Verification items for the finished model (mm, model axes). Face numbers are marked on the shaded views. A direction names the side the tool comes from. Give positions to 0.01 mm unless a question says otherwise; leave off trailing zeros. Write each loop counter-clockwise with the first axis right and the second up, starting at its lowest first coordinate (ties: lowest second). Pieces come first, ordered by that corner, then holes. Notation, with made-up numbers: (86.5, 28.5) -> (112.5, 28.5) arc R16 ccw to (112.5, 36.5) -> close; hole circle Ø11 at (42, 70). An arc over 180 degrees is marked (long way). Use one line per item in the form item = value. Start each with the question number.
(1) Depth check by flat-ended pin: pin 1 Ø5 at (x, z) = (-81.5, -1) entering from +Y; pin 2 Ø5 at (x, z) = (-165, 0) entering from -Y; pin 3 Ø4 at (y, z) = (6.5, -2) entering from +X; pin 4 Ø8 at (x, y) = (38.5, 14.5) entering from +Z. Enter the tip coordinate at first touch or a pass-through.
(2) Scan lines: L1, parallel to Z at x = -165, y = 1.9; L2, parallel to Z at x = -152, y = 7.75; L3, parallel to Y at x = -102, z = -3. Record each from-to range of solid material in increasing order.
(3) Section check C-C, the plane y = 12.25. Record the cut outline in (x, z), plus the area to 3 significant figures.
(4) Section check A-A, the plane z = 0. Record the cut outline in (x, y), plus the area to 3 significant figures.
(5) Section check B-B, the plane x = 64. Record the cut outline in (y, z).
(6) Set-up check for the marked faces 1 and 2: record each of +Z, -Z, +X, -X, +Y, -Y from which the full face is reachable in a straight line by a thin tool's end or side.
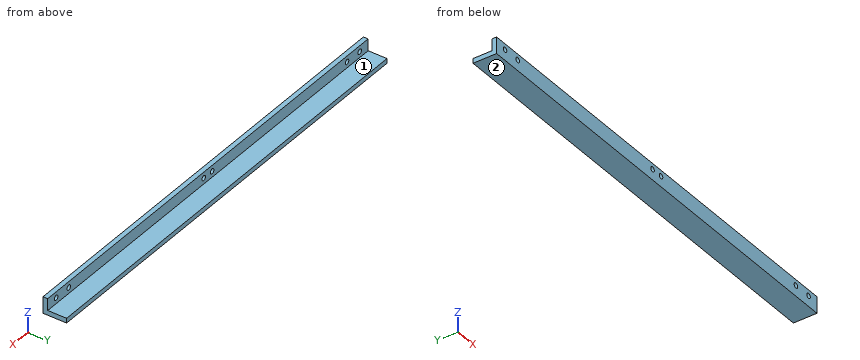
from build123d import *

# Parameters (mm, degrees)
SKETCH1_W           = 380
SKETCH1_H           = 10
SKETCH1_R           = 2.1
BOSS_EXTRUDE1_DEPTH = 4
SKETCH2_W           = 380
SKETCH2_H           = 20
BOSS_EXTRUDE2_DEPTH = 4


with BuildPart() as part:
    # Sketch1 → Boss-Extrude1 (new body)
    with BuildSketch(Plane(origin=(0, 0, 0), x_dir=(1, 0, 0), z_dir=(0, 1, 0))):
        Rectangle(SKETCH1_W, SKETCH1_H)
        with Locations(Location((-180, 0, 0), (0, 0, 270))):
            Circle(SKETCH1_R, mode=Mode.SUBTRACT)
        with Locations(Location((-165, 0, 0), (0, 0, 270))):
            Circle(SKETCH1_R, mode=Mode.SUBTRACT)
        with Locations(Location((165, 0, 0), (0, 0, 90))):
            Circle(SKETCH1_R, mode=Mode.SUBTRACT)
        with Locations(Location((180, 0, 0), (0, 0, 90))):
            Circle(SKETCH1_R, mode=Mode.SUBTRACT)
        with Locations(Location((5, 0, 0), (0, 0, 270))):
            Circle(SKETCH1_R, mode=Mode.SUBTRACT)
        with Locations(Location((-5, 0, 0), (0, 0, 270))):
            Circle(SKETCH1_R, mode=Mode.SUBTRACT)
    extrude(amount=BOSS_EXTRUDE1_DEPTH)

    # Sketch2 → Boss-Extrude2 (add)
    with BuildSketch(Plane(origin=(0, 0, -5), x_dir=(-1, 0, 0), z_dir=(0, 0, -1))):
        with Locations((0, 10)):
            Rectangle(SKETCH2_W, SKETCH2_H)
    extrude(amount=BOSS_EXTRUDE2_DEPTH)


solid = part.part
Completed:
q1.pin_1 = 4
q1.pin_2 = 0
q1.pin_3 = through
q1.pin_4 = -5
q2.L1 = -9 to -2.1, 2.1 to 5
q2.L2 = -9 to -5
q2.L3 = 0 to 4
q3.outline = (-190, -9) -> (190, -9) -> (190, -5) -> (-190, -5) -> close
q3.area = 1,520 mm²
q4.outline = (-190, 0) -> (-182.1, 0) -> (-182.1, 4) -> (-190, 4) -> close; (-177.9, 0) -> (-167.1, 0) -> (-167.1, 4) -> (-177.9, 4) -> close; (-162.9, 0) -> (-7.1, 0) -> (-7.1, 4) -> (-162.9, 4) -> close; (-2.9, 0) -> (2.9, 0) -> (2.9, 4) -> (-2.9, 4) -> close; (7.1, 0) -> (162.9, 0) -> (162.9, 4) -> (7.1, 4) -> close; (167.1, 0) -> (177.9, 0) -> (177.9, 4) -> (167.1, 4) -> close; (182.1, 0) -> (190, 0) -> (190, 4) -> (182.1, 4) -> close
q4.area = 1,420 mm²
q5.outline = (0, -9) -> (20, -9) -> (20, -5) -> (4, -5) -> (4, 5) -> (0, 5) -> close
q6.face_1 = +Z, +X, -X, +Y
q6.face_2 = -Z, +X, -X, +Y, -Y
